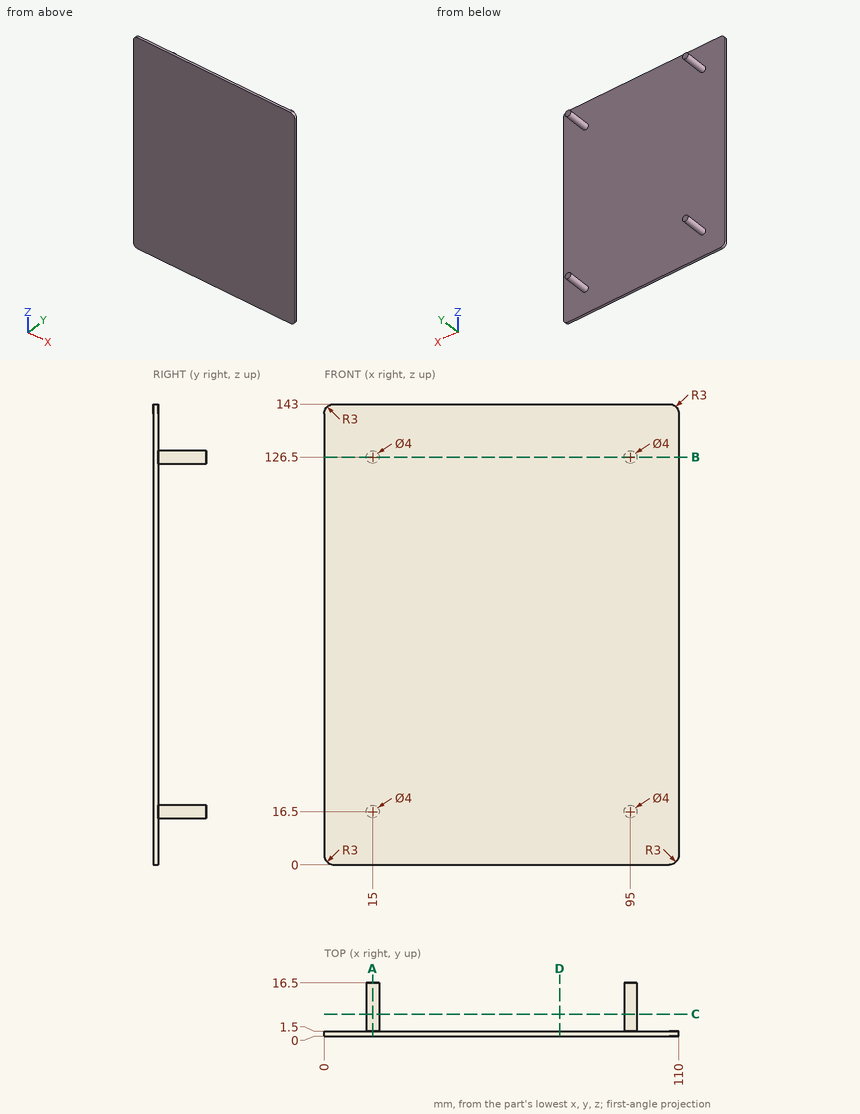
Drawing for the job (mm, zero at the part's lowest x, y, z). Coordinates: 2 decimals unless noted, no trailing zeros. Loops run counter-clockwise (first coordinate to the right, second up) from the corner with the lowest first, then second, coordinate; pieces in that order, holes last. Notation, with made-up numbers: (62.5, 83) - (69.5, 83) arc R31 ccw to (69.5, 117) - close; hole circle Ø11 at (59, 64). An arc over 180 degrees is marked (long way). Use CSV: the item, a comma, the result in double quotes. Start each with the question number.
Q1. Cut at D-D, the plane x = 73. List the corners of the cut face in (y, z), then the cut area to 4 significant figures.
Q2. Cut at C-C, the plane y = 6.75. List the corners of the cut face in (x, z), then the cut area to 3 significant figures.
Q3. Cut at A-A, the plane x = 15. List the corners of the cut face in (y, z), then the cut area to 4 significant figures.
Q4. Drop flat-ended pins along their axis: P1, Ø12, axis at x = 34.5, z = 21.5, coming from the -Y side; P2, Ø3, axis at x = 55, z = 50.5, coming from the +Y side; P3, Ø8, axis at y = 8, z = 71, coming from the -X side. Give the stop position or say it passes through.
Q5. Probe probe 1 along Z at (x, y) = (95, 9.25); probe 2 along Y at (x, z) = (82.5, 91.5); probe 3 along X at (y, z) = (12.25, 125.5). List the from-to ranges inside material, lowest first. Write a range as from..to.
Q6. Cut at B-B, the plane z = 126.5. List the corners of the cut face in (x, y).
Here are the results:
1,outline,"(0, 0) - (1.5, 0) - (1.5, 143) - (0, 143) - close"
1,area,"214.5 mm2"
2,outline,"circle Ø4 at (15, 16.5); circle Ø4 at (15, 126.5); circle Ø4 at (95, 16.5); circle Ø4 at (95, 126.5)"
2,area,"50.3 mm2"
3,outline,"(0, 0) - (1.5, 0) - (1.5, 14.5) - (16.5, 14.5) - (16.5, 18.5) - (1.5, 18.5) - (1.5, 124.5) - (16.5, 124.5) - (16.5, 128.5) - (1.5, 128.5) - (1.5, 143) - (0, 143) - close"
3,area,"334.5 mm2"
4,P1,"y = 0"
4,P2,"y = 1.5"
4,P3,"through"
5,probe 1,"14.5..18.5, 124.5..128.5"
5,probe 2,"0..1.5"
5,probe 3,"13.27..16.73, 93.27..96.73"
6,outline,"(0, 0) - (110, 0) - (110, 1.5) - (97, 1.5) - (97, 16.5) - (93, 16.5) - (93, 1.5) - (17, 1.5) - (17, 16.5) - (13, 16.5) - (13, 1.5) - (0, 1.5) - close"
